Design review of the part built by this model. Coordinates are the model's own, in mm. Face numbers are marked on the shaded views. Round coordinates to 2 decimals unless told otherwise and drop trailing zeros. Loops run counter-clockwise (first coordinate to the right, second up) from the corner with the lowest first, then second, coordinate; pieces in that order, holes last. Notation, with made-up numbers: (66, 18.25) - (120, 18.25) arc R22 cw to (120, 41.25) - close; hole circle Ø7 at (25.5, 55). An arc over 180 degrees is marked (long way). Use one line per item in the form item = value. Start each with the question number.
(1) We need section A-A, the plane z = 3. Write out the cut boundary in (x, y), then the cut area to 3 significant figures.
(2) Wall thickness on probe 1 along Y at (x, z) = (-125, 5.75); probe 2 along X at (y, z) = (121.5, 7); probe 3 along X at (y, z) = (-133.5, 7.75): over which ranges is each line inside the solid? List them lowest first. Write a range as [from, to].
(3) For pin 1 (20 mm diameter, centred on x = 125, y = 125, fed in from +Z), flat-tipped, find the tip position at first contact; note if it passes through.
(4) The part is to be moulded in two halves that separate along Z. For the marked faces 1 and 2, say which applies: released by +Z, released by -Z, zero draft, split by the parting line, or undercut.
(5) We need section B-B, the plane x = 125. Write out the cut boundary in (y, z), then the cut area to 3 significant figures.
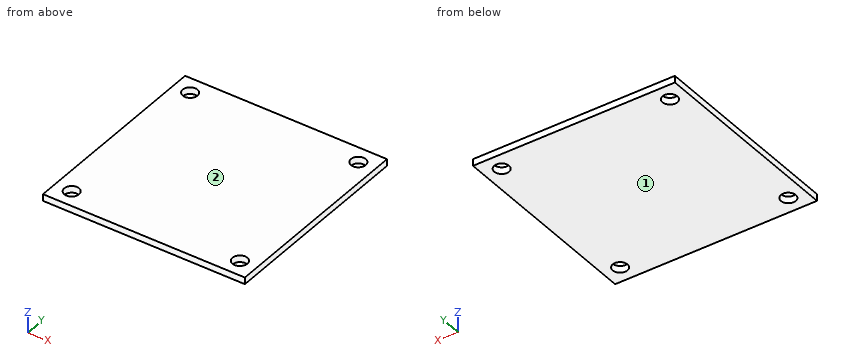
from build123d import *

# Parameters (mm, degrees)
SKETCH1_W           = 300
SKETCH1_H           = 300
SKETCH1_R           = 11
BOSS_EXTRUDE1_DEPTH = 10


with BuildPart() as part:
    # Sketch1 → Boss-Extrude1 (new body)
    with BuildSketch(Plane.XY):
        Rectangle(SKETCH1_W, SKETCH1_H)
        with Locations((-125, 125)):
            Circle(SKETCH1_R, mode=Mode.SUBTRACT)
        with Locations((125, 125)):
            Circle(SKETCH1_R, mode=Mode.SUBTRACT)
        with Locations((125, -125)):
            Circle(SKETCH1_R, mode=Mode.SUBTRACT)
        with Locations((-125, -125)):
            Circle(SKETCH1_R, mode=Mode.SUBTRACT)
    extrude(amount=BOSS_EXTRUDE1_DEPTH)


solid = part.part
Data:
q1.outline = (-150, -150) - (150, -150) - (150, 150) - (-150, 150) - close; hole circle Ø22 at (-125, -125); hole circle Ø22 at (-125, 125); hole circle Ø22 at (125, -125); hole circle Ø22 at (125, 125)
q1.area = 88,500 mm^2
q2.probe_1 = [-150, -136], [-114, 114], [136, 150]
q2.probe_2 = [-150, -135.43], [-114.57, 114.57], [135.43, 150]
q2.probe_3 = [-150, -131.98], [-118.02, 118.02], [131.98, 150]
q3.pin_1 = through
q4.face_1 = released by -Z
q4.face_2 = released by +Z
q5.outline = (-150, 0) - (-136, 0) - (-136, 10) - (-150, 10) - close; (-114, 0) - (114, 0) - (114, 10) - (-114, 10) - close; (136, 0) - (150, 0) - (150, 10) - (136, 10) - close
q5.area = 2,560 mm^2
